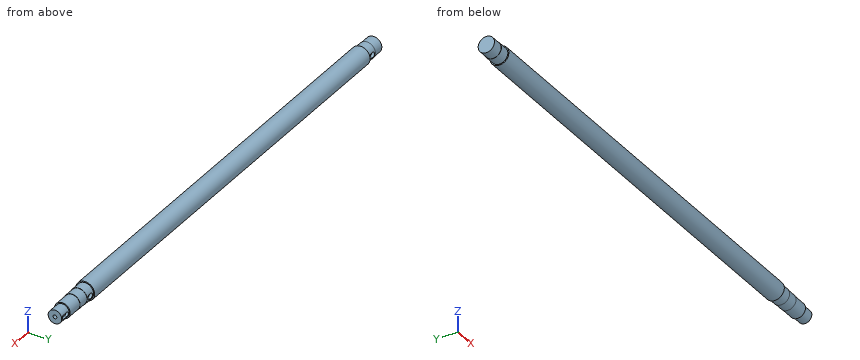
from build123d import *

# Parameters (mm, degrees)
SKETCH_1_R             = 17.5
EXTRUDE_1_DEPTH        = 410
SKETCH_2_R             = 15.5
EXTRUDE_2_DEPTH        = 19
SKETCH_3_R             = 15
EXTRUDE_3_DEPTH        = 20
SKETCH_4_R             = 14.5
EXTRUDE_4_DEPTH        = 29
SKETCH_5_R             = 12.5
EXTRUDE_5_DEPTH        = 22
CUT_EXTRUDE_1_DEPTH    = 5.83
CUT_EXTRUDE_2_DEPTH    = 7.66
HOLE_WIZARD_M8_1_D     = 6.8
HOLE_WIZARD_M8_1_DEPTH = 20
HOLE_WIZARD_M8_1_TIP   = 2.042926105


with BuildPart() as part:
    # 草图1 → 凸台-拉伸1 (new, symmetric)
    with BuildSketch(Plane(origin=(0, 0, 0), x_dir=(0, 0, -1), z_dir=(1, 0, 0))):
        with Locations(Location((0, 0, 0), (0, 0, 180))):
            Circle(SKETCH_1_R)
    extrude(amount=EXTRUDE_1_DEPTH, both=True)

    # 草图2 → 凸台-拉伸2 (add)
    with BuildSketch(Plane(origin=(410, 0, 0), x_dir=(0, 0, -1), z_dir=(1, 0, 0))):
        Circle(SKETCH_2_R)
    extrude_2 = extrude(amount=EXTRUDE_2_DEPTH)

    # 草图3 → 凸台-拉伸3 (add)
    with BuildSketch(Plane(origin=(429, 0, 0), x_dir=(0, 0, -1), z_dir=(1, 0, 0))):
        Circle(SKETCH_3_R)
    extrude_3 = extrude(amount=EXTRUDE_3_DEPTH)

    # 草图4 → 凸台-拉伸4 (add)
    with BuildSketch(Plane(origin=(449, 0, 0), x_dir=(0, 0, -1), z_dir=(1, 0, 0))):
        with Locations(Location((0, 0, 0), (0, 0, 180))):
            Circle(SKETCH_4_R)
    extrude(amount=EXTRUDE_4_DEPTH)

    # 草图5 → 凸台-拉伸5 (add)
    with BuildSketch(Plane(origin=(478, 0, 0), x_dir=(0, 0, -1), z_dir=(1, 0, 0))):
        Circle(SKETCH_5_R)
    extrude(amount=EXTRUDE_5_DEPTH)

    # 镜向1: 凸台-拉伸2, 凸台-拉伸3 across plane
    add(extrude_2.mirror(Plane(origin=(0, 0, 0), x_dir=(0, 0, 1), z_dir=(1, 0, 0))))
    add(extrude_3.mirror(Plane(origin=(0, 0, 0), x_dir=(0, 0, 1), z_dir=(1, 0, 0))))

    # 草图6 → 切除-拉伸1 (cut)
    with BuildSketch(Plane(origin=(0, 15.5, 0), x_dir=(1, 0, 0), z_dir=(0, 1, 0))):
        with BuildLine():
            Line((-418, -5), (-422, -5))
            ThreePointArc((-422, -5), (-427, 0), (-422, 5))
            Line((-422, 5), (-418, 5))
            ThreePointArc((-418, 5), (-413, 0), (-418, -5))
        make_face()
        with BuildLine():
            Line((422, -5), (418, -5))
            ThreePointArc((418, -5), (413, 0), (418, 5))
            Line((418, 5), (422, 5))
            ThreePointArc((422, 5), (427, 0), (422, -5))
        make_face()
    extrude(amount=-CUT_EXTRUDE_1_DEPTH, mode=Mode.SUBTRACT)

    # 草图7 → 切除-拉伸2 (cut)
    with BuildSketch(Plane(origin=(0, 15.5, 0), x_dir=(1, 0, 0), z_dir=(0, 1, 0))):
        with BuildLine():
            Line((484, 4), (494, 4))
            ThreePointArc((494, 4), (498, 0), (494, -4))
            Line((494, -4), (484, -4))
            ThreePointArc((484, -4), (480, 0), (484, 4))
        make_face()
    extrude(amount=-CUT_EXTRUDE_2_DEPTH, mode=Mode.SUBTRACT)

    # M8 螺纹孔1
    with Locations(Plane(origin=(500, 0, 0), x_dir=(0, 0, -1), z_dir=(1, 0, 0))):
        with Locations((0, 0)):
            Hole(HOLE_WIZARD_M8_1_D / 2, depth=HOLE_WIZARD_M8_1_DEPTH)
            with Locations((0, 0, -(HOLE_WIZARD_M8_1_DEPTH + HOLE_WIZARD_M8_1_TIP / 2))):  # 118° drill point
                Cone(0, HOLE_WIZARD_M8_1_D / 2, HOLE_WIZARD_M8_1_TIP, mode=Mode.SUBTRACT)


solid = part.part
Check sheet for the modelled part. Datum: model origin and axes. Units: mm. Round coordinates to 2 decimals unless told otherwise and drop trailing zeros. Order: outer loops, then holes, each group sorted by start corner. A loop starts at its lowest first (then second) coordinate and runs counter-clockwise, first axis right, second up.
(1) Cross-section at A-A, the plane x = -368. Enter the section's corners in (y, z), and give its area (3 significant figures).
(2) Go/stop test with flat-tipped pins: P1, Ø3, axis at x = 420.5, y = 12.5, coming from the -Z side; P2, Ø1.5, axis at x = 358.5, y = -9.5, coming from the -Z side; P3, Ø4.5, axis at x = 421, y = 12.5, coming from the +Z side. Record where each tip stops, or that it passes through.
(3) Scan lines: probe 1 along Y at (x, z) = (489.5, 0); probe 2 along X at (y, z) = (13.5, 10.5); probe 3 along X at (y, z) = (-13.5, -2). Record each from-to range of solid material in increasing order.
Check sheet entries:
1. outline: circle Ø35 at (0, 0)
1. area: 962 mm2
2. P1: stops at z = -10.92
2. P2: stops at z = -15.16
2. P3: stops at z = 11.63
3. probe 1: y = -12.5 to -3.4, 3.4 to 7.84
3. probe 2: x = -410 to 410
3. probe 3: x = -449 to 478
